CAD build for the part. Positions are in the model's coordinates, mm. Give positions to 0.01 mm unless a question says otherwise; leave off trailing zeros. Write each loop counter-clockwise with the first axis right and the second up, starting at its lowest first coordinate (ties: lowest second). Pieces come first, ordered by that corner, then holes. Notation, with made-up numbers: (-23, 54) -> (3, 54) arc R14 ccw to (3, 80) -> close; hole circle Ø11 at (7, 28). An arc over 180 degrees is marked (long way). Answer as a JSON object with one key per item and string values.
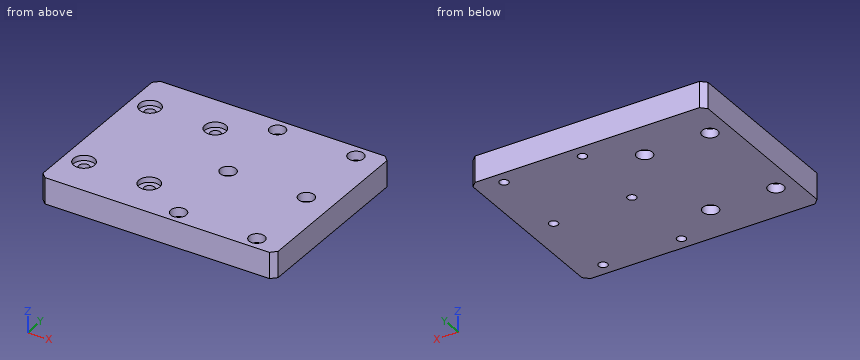
```python
from build123d import *

# Parameters (mm, degrees)
SKETCH_1_W                = 90
SKETCH_1_H                = 70
EXTRUDE_1_DEPTH           = 5
HOLE_WIZARD_1_D           = 3.4
HOLE_WIZARD_1_CBORE_D     = 6
HOLE_WIZARD_1_CBORE_DEPTH = 3.4
HOLE_WIZARD_3_D           = 3.2
HOLE_WIZARD_3_CBORE_D     = 6
HOLE_WIZARD_3_CBORE_DEPTH = 3.4
SKETCH_6_R                = 4
CUT_EXTRUDE_1_DEPTH       = 2
SKETCH_8_R                = 2
CUT_EXTRUDE_2_DEPTH       = 2
CHAMFER_1_SIZE            = 2


with BuildPart() as part:
    # 草图1 → 凸台-拉伸1 (new, symmetric)
    with BuildSketch(Plane.XY):
        Rectangle(SKETCH_1_W, SKETCH_1_H)
    extrude(amount=EXTRUDE_1_DEPTH, both=True)

    # 打孔尺寸(%根据)内六角圆柱头螺钉的类型1 (through all)
    with Locations(Plane.XY.offset(5)):
        with Locations((5, 30), (5, 0), (5, -30), (35, 30), (35, 0), (35, -30)):
            CounterBoreHole(HOLE_WIZARD_1_D / 2, HOLE_WIZARD_1_CBORE_D / 2, HOLE_WIZARD_1_CBORE_DEPTH)

    # 打孔尺寸(%根据)内六角圆柱头螺钉的类型3 (through all)
    with Locations(Plane(origin=(0, 0, -5), x_dir=(-1, 0, 0), z_dir=(0, 0, -1))):
        with Locations((37.5, 20), (12.5, 20), (12.5, -20), (37.5, -20)):
            CounterBoreHole(HOLE_WIZARD_3_D / 2, HOLE_WIZARD_3_CBORE_D / 2, HOLE_WIZARD_3_CBORE_DEPTH)

    # 草图6 → 切除-拉伸1 (cut)
    with BuildSketch(Plane.XY.offset(5)):
        with Locations((-37.5, 20)):
            Circle(SKETCH_6_R)
        with Locations((-12.5, 20)):
            Circle(SKETCH_6_R)
        with Locations((-37.5, -20)):
            Circle(SKETCH_6_R)
        with Locations((-12.5, -20)):
            Circle(SKETCH_6_R)
    extrude(amount=-CUT_EXTRUDE_1_DEPTH, mode=Mode.SUBTRACT)

    # 草图8 → 切除-拉伸2 (cut)
    with BuildSketch(Plane.XY.offset(3)):
        with Locations((-37.5, 20)):
            Circle(SKETCH_8_R)
        with Locations((-37.5, -20)):
            Circle(SKETCH_8_R)
        with Locations((-12.5, -20)):
            Circle(SKETCH_8_R)
        with Locations((-12.5, 20)):
            Circle(SKETCH_8_R)
    extrude(amount=-CUT_EXTRUDE_2_DEPTH, mode=Mode.SUBTRACT)

    # 倒角1
    chamfer_1_edges = [part.edges().sort_by_distance(p)[0] for p in [
        (45, -35, 0),
        (-45, -35, 0),
        (-45, 35, 0),
        (45, 35, 0),
    ]]
    chamfer(chamfer_1_edges, length=CHAMFER_1_SIZE)


solid = part.part
```
1) Pin check, flat tips, straight feed: pin 1 (5.5 mm diameter, centred on x = 5, y = -30, fed in from +Z); pin 2 (5.5 mm diameter, centred on x = -37.5, y = -20, fed in from +Z); pin 3 (1.8 mm diameter, centred on x = -14, y = -19, fed in from -Z). Stop position of each tip, or through.
Model answer:
{"pin 1": "stops at z = 1.6", "pin 2": "stops at z = 3", "pin 3": "stops at z = -1.6"}
2) Slice it at B-B (z = -3.5). State how many separate pieces and enclosed holes the cut face has, then the cut area to 3 significant figures.
Model answer:
{"separate pieces": "1", "enclosed holes": "10", "area": "6,120 mm2"}
3) Slice it at C-C (y = -30). List the corners of the cut face in (x, z).
Model answer:
{"outline": "(-45, -5) -> (3.3, -5) -> (3.3, 1.6) -> (2, 1.6) -> (2, 5) -> (-45, 5) -> close; (6.7, -5) -> (33.3, -5) -> (33.3, 1.6) -> (32, 1.6) -> (32, 5) -> (8, 5) -> (8, 1.6) -> (6.7, 1.6) -> close; (36.7, -5) -> (45, -5) -> (45, 5) -> (38, 5) -> (38, 1.6) -> (36.7, 1.6) -> close"}
4) Wall check: probe 1 along Y at (x, z) = (-12.5, 4.5); probe 2 along X at (y, z) = (-29.5, -3.75); probe 3 along Z at (x, y) = (7, -31.5). Give the ranges that are in metal, low to high.
Model answer:
{"probe 1": "y = -35 to -24, -16 to 16, 24 to 35", "probe 2": "x = -45 to 3.38, 6.62 to 33.38, 36.62 to 45", "probe 3": "z = -5 to 1.6"}
5) Slice it at A-A (x = 5). List the corners of the cut face in (y, z), then the cut area to 3 significant figures.
Model answer:
{"outline": "(-35, -5) -> (-31.7, -5) -> (-31.7, 1.6) -> (-33, 1.6) -> (-33, 5) -> (-35, 5) -> close; (-28.3, -5) -> (-1.7, -5) -> (-1.7, 1.6) -> (-3, 1.6) -> (-3, 5) -> (-27, 5) -> (-27, 1.6) -> (-28.3, 1.6) -> close; (1.7, -5) -> (28.3, -5) -> (28.3, 1.6) -> (27, 1.6) -> (27, 5) -> (3, 5) -> (3, 1.6) -> (1.7, 1.6) -> close; (31.7, -5) -> (35, -5) -> (35, 5) -> (33, 5) -> (33, 1.6) -> (31.7, 1.6) -> close", "area": "571 mm2"}
